Could you check a few things on this model? Use its own coordinates, in mm. Give positions to 0.01 mm unless a question says otherwise; leave off trailing zeros. Loops run counter-clockwise (first coordinate to the right, second up) from the corner with the lowest first, then second, coordinate; pieces in that order, holes last.
1. Imagine slicing it at C-C (z = 2.25). List the corners of the cut face in (x, y) for me.
2. I need wall thicknesses on line 1 along Y through (x, z) = (0, 4); line 2 along X through (y, z) = (44.5, 7.5). Which ranges of each line are inside material? Lowest first, please.
3. Thinking about a two-plate mould opening in X: for faces 1 (the flat face through (0, 1, 0)), 2 (the flat face through (-25, -1, 4)), 3 (the cylindrical face through (-2.4, 35.5, 3.9)), which applies, +X half, -X half, draft (parallel to the pull), parting line (faces both ways), or undercut?
4. Imagine slicing it at A-A (x = 0). List the corners of the cut face in (y, z) for me.
5. Imagine slicing it at B-B (y = 40). List the corners of the cut face in (x, z) for me, plus the area to 3 significant figures.
```python
from build123d import *

# Parameters (mm, degrees)
SKETCH1_W              = 50
SKETCH1_H              = 130
BOSS_EXTRUDE1_DEPTH    = 8
M12_TAPPED_HOLE1_D     = 10.2
M12_TAPPED_HOLE1_DEPTH = 29.25
M12_TAPPED_HOLE1_TIP   = 3.064389157


with BuildPart() as part:
    # Sketch1 → Boss-Extrude1 (new body)
    with BuildSketch(Plane.XY):
        Rectangle(SKETCH1_W, SKETCH1_H)
    extrude(amount=BOSS_EXTRUDE1_DEPTH)

    # M12 Tapped Hole1
    with Locations(Plane.XY.offset(8)):
        with Locations((0, 40), (0, -40)):
            Hole(M12_TAPPED_HOLE1_D / 2, depth=M12_TAPPED_HOLE1_DEPTH)
            with Locations((0, 0, -(M12_TAPPED_HOLE1_DEPTH + M12_TAPPED_HOLE1_TIP / 2))):  # 118° drill point
                Cone(0, M12_TAPPED_HOLE1_D / 2, M12_TAPPED_HOLE1_TIP, mode=Mode.SUBTRACT)


solid = part.part
```
Derived:
1. outline: (-25, -65) - (25, -65) - (25, 65) - (-25, 65) - close; hole circle Ø10.2 at (0, -40); hole circle Ø10.2 at (0, 40)
2. line 1: y = -65 to -45.1, -34.9 to 34.9, 45.1 to 65
2. line 2: x = -25 to -2.4, 2.4 to 25
3. face 1: draft
3. face 2: -X half
3. face 3: undercut
4. outline: (-65, 0) - (-45.1, 0) - (-45.1, 8) - (-65, 8) - close; (-34.9, 0) - (34.9, 0) - (34.9, 8) - (-34.9, 8) - close; (45.1, 0) - (65, 0) - (65, 8) - (45.1, 8) - close
5. outline: (-25, 0) - (-5.1, 0) - (-5.1, 8) - (-25, 8) - close; (5.1, 0) - (25, 0) - (25, 8) - (5.1, 8) - close
5. area: 318 mm2
